Source: CAD feature listing. Evaluate the final solid. Frame: model axes, mm. Give positions to 0.01 mm unless a question says otherwise; leave off trailing zeros. Write each loop counter-clockwise with the first axis right and the second up, starting at its lowest first coordinate (ties: lowest second). Pieces come first, ordered by that corner, then holes.
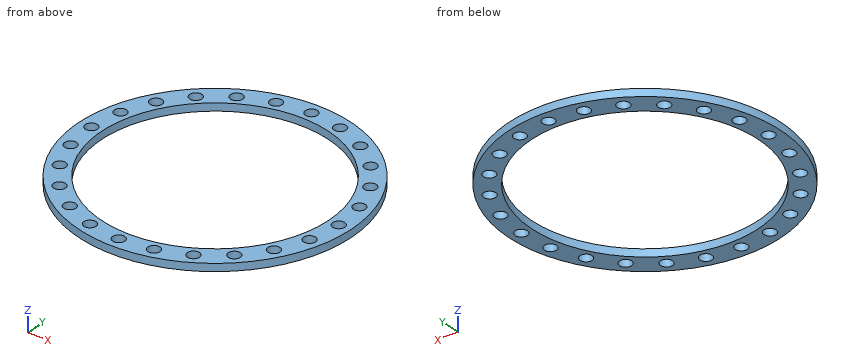
```python
from build123d import *

# Parameters (mm, degrees)
SKETCH_1_R          = 450
EXTRUDE_1_DEPTH     = 25
SKETCH_2_R          = 20
CUT_EXTRUDE_1_DEPTH = 34
SKETCH_3_R          = 375
CUT_EXTRUDE_2_DEPTH = 420


with BuildPart() as part:
    # 草图1 → 凸台-拉伸1 (new body)
    with BuildSketch(Plane.XY):
        Circle(SKETCH_1_R)
    extrude(amount=EXTRUDE_1_DEPTH)

    # 草图2 → 切除-拉伸1 (cut)
    with BuildSketch(Plane.XY.offset(25)):
        with Locations((0, 410)):
            Circle(SKETCH_2_R)
        with Locations((106.115808492, 396.029588779)):
            Circle(SKETCH_2_R)
        with Locations((205, 355.070415552)):
            Circle(SKETCH_2_R)
        with Locations((289.913780286, 289.913780286)):
            Circle(SKETCH_2_R)
        with Locations((355.070415552, 205)):
            Circle(SKETCH_2_R)
        with Locations((396.029588779, 106.115808492)):
            Circle(SKETCH_2_R)
        with Locations((410, 0)):
            Circle(SKETCH_2_R)
        with Locations((396.029588779, -106.115808492)):
            Circle(SKETCH_2_R)
        with Locations((355.070415552, -205)):
            Circle(SKETCH_2_R)
        with Locations((289.913780286, -289.913780286)):
            Circle(SKETCH_2_R)
        with Locations((205, -355.070415552)):
            Circle(SKETCH_2_R)
        with Locations((106.115808492, -396.029588779)):
            Circle(SKETCH_2_R)
        with Locations((0, -410)):
            Circle(SKETCH_2_R)
        with Locations((-106.115808492, -396.029588779)):
            Circle(SKETCH_2_R)
        with Locations((-205, -355.070415552)):
            Circle(SKETCH_2_R)
        with Locations((-289.913780286, -289.913780286)):
            Circle(SKETCH_2_R)
        with Locations((-355.070415552, -205)):
            Circle(SKETCH_2_R)
        with Locations((-396.029588779, -106.115808492)):
            Circle(SKETCH_2_R)
        with Locations((-410, 0)):
            Circle(SKETCH_2_R)
        with Locations((-396.029588779, 106.115808492)):
            Circle(SKETCH_2_R)
        with Locations((-355.070415552, 205)):
            Circle(SKETCH_2_R)
        with Locations((-289.913780286, 289.913780286)):
            Circle(SKETCH_2_R)
        with Locations((-205, 355.070415552)):
            Circle(SKETCH_2_R)
        with Locations((-106.115808492, 396.029588779)):
            Circle(SKETCH_2_R)
    extrude(amount=-CUT_EXTRUDE_1_DEPTH, mode=Mode.SUBTRACT)

    # 草图3 → 切除-拉伸2 (cut)
    with BuildSketch(Plane.XY.offset(25)):
        Circle(SKETCH_3_R)
    extrude(amount=-CUT_EXTRUDE_2_DEPTH, mode=Mode.SUBTRACT)


solid = part.part
```
1. Section query C-C (x = 205). Return loops of the section in (y, z).
2. Pin query (flat end, axial travel): P1, Ø10, axis at x = -292.5, z = 2.5, coming from the +Y side; P2, Ø2, axis at y = -65, z = 15, coming from the +X side; P3, Ø24, axis at x = 396.03, y = -106.12, coming from the +Z side; P4, Ø8, axis at x = 113.5, z = 18, coming from the +Y side. Return the tip coordinate at first contact, or that it passes through.
3. Section query D-D (z = 10.5). Give the number of separate pieces and of enclosed holes in the cut face, plus the area to 3 significant figures.
4. Section query B-B (y = -246). Return loops of the section in (x, z), plus the area to 3 significant figures.
5. Section query A-A (x = 54.5). Return loops of the section in (y, z), plus the area to 3 significant figures.
6. Line query: probe 1 along Y at (x, z) = (0.5, 14); probe 2 along Y at (x, z) = (-205, 6.5); probe 3 along X at (y, z) = (-401.5, 18.75). Output: solid intervals per line, ascending.
The answers:
1. outline: (-400.59, 0) - (-375.07, 0) - (-375.07, 25) - (-400.59, 25) - close; (-335.07, 0) - (-314.01, 0) - (-314.01, 25) - (-335.07, 25) - close; (314.01, 0) - (335.07, 0) - (335.07, 25) - (314.01, 25) - close; (375.07, 0) - (400.59, 0) - (400.59, 25) - (375.07, 25) - close
2. P1: stops at y = 346.18
2. P2: stops at x = 445.43
2. P3: passes through
2. P4: stops at y = 436.47
3. separate pieces: 1
3. enclosed holes: 25
3. area: 164,000 mm2
4. outline: (-376.81, 0) - (-283.04, 0) - (-283.04, 25) - (-376.81, 25) - close; (283.04, 0) - (376.81, 0) - (376.81, 25) - (283.04, 25) - close
4. area: 4,690 mm2
5. outline: (-446.69, 0) - (-371.02, 0) - (-371.02, 25) - (-446.69, 25) - close; (371.02, 0) - (446.69, 0) - (446.69, 25) - (371.02, 25) - close
5. area: 3,780 mm2
6. probe 1: y = -450 to -429.99, -390.01 to -375, 375 to 390.01, 429.99 to 450
6. probe 2: y = -400.59 to -375.07, -335.07 to -314.01, 314.01 to 335.07, 375.07 to 400.59
6. probe 3: x = -203.22 to -125.35, -86.88 to -18.1, 18.1 to 86.88, 125.35 to 203.22
